The listing builds one solid part. Answer for the finished solid, in the listing's coordinates (mm). Round coordinates to 2 decimals unless told otherwise and drop trailing zeros. Write each loop counter-clockwise with the first axis right and the second up, starting at its lowest first coordinate (ties: lowest second). Pieces come first, ordered by that corner, then holes. Notation, with made-up numbers: M -26,-8 L 14,-8 A8 cw 14,-2 Z; hole C 24.25,-28 d11. An arc over 180 degrees is marked long. Write each question's results on one line, items separated by ' | '.
from build123d import *

# Parameters (mm, degrees)
SKETCH1_W                 = 20
SKETCH1_H                 = 90
BOSS_EXTRUDE1_DEPTH       = 15
CHAMFER1_SIZE             = 5
CUT_EXTRUDE1_DEPTH        = 49.476798574
CUT_EXTRUDE2_DEPTH        = 49.476798574
CUT_EXTRUDE3_DEPTH        = 6
LINEAR_PATTERN1_COUNT     = 2
LINEAR_PATTERN1_PITCH     = 30
LINEAR_PATTERN1_COL_COUNT = 2
LINEAR_PATTERN1_COL_PITCH = 30


with BuildPart() as part:
    # Sketch1 → Boss-Extrude1 (new body)
    with BuildSketch(Plane(origin=(0, 0, 0), x_dir=(1, 0, 0), z_dir=(0, 1, 0))):
        Rectangle(SKETCH1_W, SKETCH1_H)
    extrude(amount=BOSS_EXTRUDE1_DEPTH)

    # Chamfer1
    chamfer1_edges = [part.edges().sort_by_distance(p)[0] for p in [
        (-10, 15, 0),
    ]]
    chamfer(chamfer1_edges, length=CHAMFER1_SIZE)

    # Sketch2 → Cut-Extrude1 (cut, through all)
    with BuildSketch(Plane(origin=(0, 15, 0), x_dir=(1, 0, 0), z_dir=(0, 1, 0))):
        Polygon((10, 25), (9, 45), (10, 45), align=None)
    extrude(amount=-CUT_EXTRUDE1_DEPTH, mode=Mode.SUBTRACT)

    # Sketch3 → Cut-Extrude2 (cut, through all)
    with BuildSketch(Plane(origin=(0, 15, 0), x_dir=(1, 0, 0), z_dir=(0, 1, 0))):
        with BuildLine():
            Line((0, 2.25), (6, 2.25))
            ThreePointArc((6, 2.25), (8.25, 0), (6, -2.25))
            Line((6, -2.25), (0, -2.25))
            ThreePointArc((0, -2.25), (-2.25, 0), (0, 2.25))
        make_face()
    cut_extrude2 = extrude(amount=-CUT_EXTRUDE2_DEPTH, mode=Mode.SUBTRACT)

    # Sketch4 → Cut-Extrude3 (cut)
    with BuildSketch(Plane(origin=(0, 15, 0), x_dir=(1, 0, 0), z_dir=(0, 1, 0))):
        with BuildLine():
            Line((0, -3.75), (6, -3.75))
            ThreePointArc((6, -3.75), (9.75, 0), (6, 3.75))
            Line((6, 3.75), (0, 3.75))
            ThreePointArc((0, 3.75), (-3.75, 0), (0, -3.75))
        make_face()
    cut_extrude3 = extrude(amount=-CUT_EXTRUDE3_DEPTH, mode=Mode.SUBTRACT)

    # Linear pattern1: Cut-Extrude2, Cut-Extrude3 ×2
    with Locations(*[(0, 0, i * LINEAR_PATTERN1_PITCH) for i in range(1, LINEAR_PATTERN1_COUNT)]):
        add(cut_extrude2, mode=Mode.SUBTRACT)
        add(cut_extrude3, mode=Mode.SUBTRACT)

    # Linear pattern1 col: Cut-Extrude2, Cut-Extrude3 ×2
    with Locations(*[(0, 0, -i * LINEAR_PATTERN1_COL_PITCH) for i in range(1, LINEAR_PATTERN1_COL_COUNT)]):
        add(cut_extrude2, mode=Mode.SUBTRACT)
        add(cut_extrude3, mode=Mode.SUBTRACT)


solid = part.part
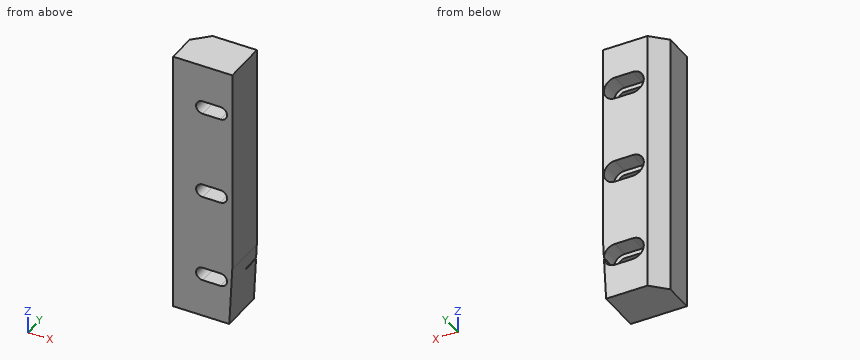
1) Section A-A (y = 3) is taken. Determine the outline of the cut face in (x, z), then the cut area to 3 significant figures.
Return value:
outline: M -10,-45 L 9,-45 L 10,-25 L 10,45 L -10,45 Z; hole M 0,-32.25 L 6,-32.25 A2.25 ccw 6,-27.75 L 0,-27.75 A2.25 ccw Z; hole M 0,-2.25 L 6,-2.25 A2.25 ccw 6,2.25 L 0,2.25 A2.25 ccw Z; hole M 0,27.75 L 6,27.75 A2.25 ccw 6,32.25 L 0,32.25 A2.25 ccw Z | area: 1,660 mm²
2) Section D-D (z = -16.5) is taken. Determine the outline of the cut face in (x, y), then the cut area to 4 significant figures.
Return value:
outline: M -10,0 L 10,0 L 10,15 L -5,15 L -10,10 Z | area: 287.5 mm²
3) Each of these flat-tipped pins is pushed along its axis until it touches: pin 1 (6 mm diameter, centred on y = 3.5, z = -30.5, fed in from +X) (3 decimals); pin 2 (4 mm diameter, centred on x = 2, z = -1, fed in from +Y); pin 3 (2 mm diameter, centred on x = 4, z = -29, fed in from +Y). Where does it stop, or does it pass through?
Return value:
pin 1: x = 9.875 | pin 2: y = 9 | pin 3: through
4) Section B-B (x = 1.5) is taken. Determine the outline of the cut face in (y, z), then the cut area to 3 significant figures.
Return value:
outline: M 0,-45 L 15,-45 L 15,-33.75 L 9,-33.75 L 9,-32.25 L 0,-32.25 Z; M 0,-27.75 L 9,-27.75 L 9,-26.25 L 15,-26.25 L 15,-3.75 L 9,-3.75 L 9,-2.25 L 0,-2.25 Z; M 0,2.25 L 9,2.25 L 9,3.75 L 15,3.75 L 15,26.25 L 9,26.25 L 9,27.75 L 0,27.75 Z; M 0,32.25 L 9,32.25 L 9,33.75 L 15,33.75 L 15,45 L 0,45 Z | area: 1,090 mm²
5) Section C-C (z = 30) is taken. Determine the outline of the cut face in (x, y), then the cut area to 3 significant figures.
Return value:
outline: M -10,0 L -2.25,0 L -2.25,9 L -3.75,9 L -3.75,15 L -5,15 L -10,10 Z; M 8.25,0 L 10,0 L 10,15 L 9.75,15 L 9.75,9 L 8.25,9 Z | area: 112 mm²
6) Find the intervals of material crossed by line 1 (Z direction, x = 1.5, y = 7); line 2 (Z direction, x = -1.75, y = 8); line 3 (X direction, y = 11.5, z = 0), in increasing order.
Return value:
line 1: -45 to -32.25, -27.75 to -2.25, 2.25 to 27.75, 32.25 to 45 | line 2: -45 to -31.41, -28.59 to -1.41, 1.41 to 28.59, 31.41 to 45 | line 3: -8.5 to -3.75, 9.75 to 10
